Geometry check sheet. Reference: the model listing, model coordinates, mm. A direction names the side the tool comes from. Coordinates: 2 decimals unless noted, no trailing zeros. Write each loop counter-clockwise with the first axis right and the second up, starting at its lowest first coordinate (ties: lowest second). Pieces come first, ordered by that corner, then holes. Notation, with made-up numbers: M -30.5,86 L -24.5,86 A11 ccw -24.5,104 Z; hole C 77.25,73.25 d5. An arc over 180 degrees is marked long. Put each result on its own line as item: value. Start each with the question number.
1) Cross-section at B-B on y = 0. Record the cut outline in (x, z).
2) Scan lines: line 1 along Y through (x, z) = (0, 1.5); line 2 along X through (y, z) = (-10.5, 0.5); line 3 along Y through (x, z) = (6, 0.9). Record each from-to range of solid material in increasing order.
3) Mould release check, pull along X, two halves, no side actions. Record for faces 4 (the flat face through (58.515, -5.991, 1.479)), 5 (the flat face through (25, -2, 3)), 6 (the cylindrical face through (-1.08, -4.88, 1.52)), 7 (the flat face through (40.58, -11.944, 1.479)): released by +X, released by -X, zero draft, split by the parting line, or undercut.
4) Gauge pin test, flat ends, axial feed: pin 1 (8 mm diameter, centred on x = 0, y = 0, fed in from +Z); pin 2 (1.5 mm diameter, centred on y = -9, z = 1.5, fed in from -X); pin 3 (1.5 mm diameter, centred on x = 10, z = 1, fed in from -Y). Record the tip position at first contact, or that the pin passes through.
5) Set-up check for faces 1 (the flat face through (11, -10, 1)), 2 (the flat face through (37.806, -11.851, 1.479)), 3 (the flat face through (54.58, -11.944, 1.479)): record each of +Z, -Z, +X, -X, +Y, -Y from which the full face is reachable in a straight line by a thin tool's end or side.
6) Cross-section at C-C on x = 9. Record the cut outline in (y, z).
7) Cross-section at D-D on y = -9. Record the cut outline in (x, z).
from build123d import *

# Parameters (mm, degrees)
BOSS_EXTRUDE3_DEPTH = 3
SKETCH4_R           = 5
CUT_EXTRUDE1_DEPTH  = 3


with BuildPart() as part:
    # Sketch3 → Boss-Extrude3 (new body)
    with BuildSketch(Plane.XY):
        with BuildLine():
            Line((0, -10), (21.747859728, -10))
            ThreePointArc((21.747859728, -10), (21.939201445, -10.038060234), (22.101413119, -10.146446609))
            Line((22.101413119, -10.146446609), (25.558597985, -13.603631476))
            Line((25.558597985, -13.603631476), (27.630628855, -10.237878069))
            ThreePointArc((27.630628855, -10.237878069), (27.81254922, -10.063502024), (28.056412947, -10))
            Line((28.056412947, -10), (28.747859728, -10))
            ThreePointArc((28.747859728, -10), (28.939201445, -10.038060234), (29.101413119, -10.146446609))
            Line((29.101413119, -10.146446609), (32.558597985, -13.603631476))
            Line((32.558597985, -13.603631476), (34.630628855, -10.237878069))
            ThreePointArc((34.630628855, -10.237878069), (34.81254922, -10.063502024), (35.056412947, -10))
            Line((35.056412947, -10), (35.747859728, -10))
            ThreePointArc((35.747859728, -10), (35.939201445, -10.038060234), (36.101413119, -10.146446609))
            Line((36.101413119, -10.146446609), (39.558597985, -13.603631476))
            Line((39.558597985, -13.603631476), (41.630628855, -10.237878069))
            ThreePointArc((41.630628855, -10.237878069), (41.81254922, -10.063502024), (42.056412947, -10))
            Line((42.056412947, -10), (42.747859728, -10))
            ThreePointArc((42.747859728, -10), (42.939201445, -10.038060234), (43.101413119, -10.146446609))
            Line((43.101413119, -10.146446609), (46.558597985, -13.603631476))
            Line((46.558597985, -13.603631476), (48.630628855, -10.237878069))
            ThreePointArc((48.630628855, -10.237878069), (48.81254922, -10.063502024), (49.056412947, -10))
            Line((49.056412947, -10), (49.747859728, -10))
            ThreePointArc((49.747859728, -10), (49.939201445, -10.038060234), (50.101413119, -10.146446609))
            Line((50.101413119, -10.146446609), (53.558597985, -13.603631476))
            Line((53.558597985, -13.603631476), (55.630628855, -10.237878069))
            ThreePointArc((55.630628855, -10.237878069), (55.81254922, -10.063502024), (56.056412947, -10))
            Line((56.056412947, -10), (56.612992327, -10))
            ThreePointArc((56.612992327, -10), (56.895260585, -9.912704047), (57.078965337, -9.681298521))
            Line((57.078965337, -9.681298521), (59.991284364, -2.196063373))
            ThreePointArc((59.991284364, -2.196063373), (59.984936133, -1.454957765), (59.470177564, -0.921758518))
            ThreePointArc((59.470177564, -0.921758518), (30.305424132, 8.170460374), (-0.189011515, 9.998213573))
            ThreePointArc((-0.189011515, 9.998213573), (-9.999553383, -0.094509978), (0, -10))
        make_face()
    extrude(amount=BOSS_EXTRUDE3_DEPTH)

    # Sketch4 → Cut-Extrude1 (cut)
    with BuildSketch(Plane.XY.offset(3)):
        Circle(SKETCH4_R)
    extrude(amount=-CUT_EXTRUDE1_DEPTH, mode=Mode.SUBTRACT)


solid = part.part
Answer key:
1. outline: M -10,0 L -5,0 L -5,3 L -10,3 Z; M 5,0 L 57.37,0 L 57.37,3 L 5,3 Z
2. line 1: y = -10 to -5, 5 to 10.01
2. line 2: x = 22.45 to 27.47, 29.45 to 34.47, 36.45 to 41.47, 43.45 to 48.47, 50.45 to 55.47
2. line 3: y = -10 to 10.23
3. face 4: released by +X
3. face 5: zero draft
3. face 6: undercut
3. face 7: undercut
4. pin 1: passes through
4. pin 2: stops at x = -5.65
4. pin 3: stops at y = -10
5. face 1: +Z, -Z, -X, -Y
5. face 2: +Z, -Z, -Y
5. face 3: +Z, -Z, +X, -Y
6. outline: M -10,0 L 10.23,0 L 10.23,3 L -10,3 Z
7. outline: M -4.36,0 L 57.34,0 L 57.34,3 L -4.36,3 Z
